For this review, take the finished solid that the model builds, in its own axes (mm). A direction names the side the tool comes from. Give positions to 0.01 mm unless a question says otherwise; leave off trailing zeros. Order: outer loops, then holes, each group sorted by start corner. A loop starts at its lowest first (then second) coordinate and runs counter-clockwise, first axis right, second up.
from build123d import *

# Parameters (mm, degrees)
SKETCH_1_W                   = 210
SKETCH_1_H                   = 60
EXTRUDE_1_DEPTH              = 12
SKETCH_2_R                   = 12.5
CUT_EXTRUDE_1_DEPTH          = 12
HOLE_WIZARD_M8_1_D           = 8.4
HOLE_WIZARD_M8_1_CBORE_D     = 15
HOLE_WIZARD_M8_1_CBORE_DEPTH = 8.6
HOLE_WIZARD_M6_2_D           = 6.4
HOLE_WIZARD_M6_2_CBORE_D     = 11
HOLE_WIZARD_M6_2_CBORE_DEPTH = 6.4
CHAMFER_1_SIZE               = 1
HOLE_WIZARD_9_0_9_1_D        = 9
SKETCH_14_W                  = 30
SKETCH_14_H                  = 20
EXTRUDE_2_DEPTH              = 12


with BuildPart() as part:
    # 草图1 → 凸台-拉伸1 (new body)
    with BuildSketch(Plane.XY):
        with Locations((105, 30)):
            Rectangle(SKETCH_1_W, SKETCH_1_H)
    extrude(amount=EXTRUDE_1_DEPTH)

    # 草图2 → 切除-拉伸1 (cut)
    with BuildSketch(Plane.XY.offset(12)):
        with Locations((105, 25)):
            Circle(SKETCH_2_R)
    extrude(amount=-CUT_EXTRUDE_1_DEPTH, mode=Mode.SUBTRACT)

    # M8 六角凹头螺钉的柱形沉头孔1 (through all)
    with Locations(Plane(origin=(0, 0, 0), x_dir=(-1, 0, 0), z_dir=(0, 0, -1))):
        with Locations((-55, 21), (-155, 21)):
            CounterBoreHole(HOLE_WIZARD_M8_1_D / 2, HOLE_WIZARD_M8_1_CBORE_D / 2, HOLE_WIZARD_M8_1_CBORE_DEPTH)

    # M6 六角凹头螺钉的柱形沉头孔2 (through all)
    with Locations(Plane.XY.offset(12)):
        with Locations((122, 42), (88, 42), (122, 8), (88, 8)):
            CounterBoreHole(HOLE_WIZARD_M6_2_D / 2, HOLE_WIZARD_M6_2_CBORE_D / 2, HOLE_WIZARD_M6_2_CBORE_DEPTH)

    # 倒角1
    chamfer_1_edges = [part.edges().sort_by_distance(p)[0] for p in [
        (210, 30, 12),
        (0, 30, 12),
        (210, 30, 0),
        (0, 30, 0),
    ]]
    chamfer(chamfer_1_edges, length=CHAMFER_1_SIZE)

    # Ø9.0 (9) 直径孔1 (through all)
    with Locations(Plane(origin=(0, 0, 0), x_dir=(-1, 0, 0), z_dir=(0, 0, -1))):
        with Locations((-192.5, 35), (-17.5, 35)):
            Hole(HOLE_WIZARD_9_0_9_1_D / 2)

    # 草图14 → 凸台-拉伸2 (add)
    with BuildSketch(Plane(origin=(0, 0, 0), x_dir=(-1, 0, 0), z_dir=(0, 0, -1))):
        with Locations((-105, -10)):
            Rectangle(SKETCH_14_W, SKETCH_14_H)
    extrude(amount=-EXTRUDE_2_DEPTH)


solid = part.part
1) We need section D-D on y = -10. Give the boundary of the cut face in (x, z).
Answer sheet:
outline: (90, 0) - (120, 0) - (120, 12) - (90, 12) - close
2) To check wall thickness, follow line 1 (Y direction, x = 122, z = 2.3); line 2 (Y direction, x = 155, z = 3.25); line 3 (Y direction, x = 127, z = 8). State the ranges of each line that lie inside material, in increasing order.
Answer sheet:
line 1: y = 0 to 4.8, 11.2 to 38.8, 45.2 to 60
line 2: y = 0 to 13.5, 28.5 to 60
line 3: y = 0 to 5.71, 10.29 to 39.71, 44.29 to 60
3) We need section B-B on y = 8. Give the boundary of the cut face in (x, z), then the cut area to 3 significant figures.
Answer sheet:
outline: (0, 1) - (1, 0) - (84.8, 0) - (84.8, 5.6) - (82.5, 5.6) - (82.5, 12) - (1, 12) - (0, 11) - close; (91.2, 0) - (118.8, 0) - (118.8, 5.6) - (116.5, 5.6) - (116.5, 12) - (93.5, 12) - (93.5, 5.6) - (91.2, 5.6) - close; (125.2, 0) - (209, 0) - (210, 1) - (210, 11) - (209, 12) - (127.5, 12) - (127.5, 5.6) - (125.2, 5.6) - close
area: 2,310 mm2
4) Clearance check with flat-ended pins moving along their axes: pin 1 (4.5 mm diameter, centred on x = 155.5, y = 17.5, fed in from -Z); pin 2 (2 mm diameter, centred on y = -8, z = 3.5, fed in from -X); pin 3 (6 mm diameter, centred on x = 166.5, z = 3.5, fed in from -Y). State where each tip first meets the part, or that it passes through.
Answer sheet:
pin 1: stops at z = 8.6
pin 2: stops at x = 90
pin 3: stops at y = 0
5) We need section A-A on x = 88. Give the boundary of the cut face in (y, z), then the cut area to 3 significant figures.
Answer sheet:
outline: (0, 0) - (4.8, 0) - (4.8, 5.6) - (2.5, 5.6) - (2.5, 12) - (0, 12) - close; (11.2, 0) - (38.8, 0) - (38.8, 5.6) - (36.5, 5.6) - (36.5, 12) - (13.5, 12) - (13.5, 5.6) - (11.2, 5.6) - close; (45.2, 0) - (60, 0) - (60, 12) - (47.5, 12) - (47.5, 5.6) - (45.2, 5.6) - close
area: 508 mm2
6) We need section C-C on x = 192.5. Give the boundary of the cut face in (y, z).
Answer sheet:
outline: (0, 0) - (30.5, 0) - (30.5, 12) - (0, 12) - close; (39.5, 0) - (60, 0) - (60, 12) - (39.5, 12) - close
7) Tool access review of faces 1 (the face through (116.505, 8.242, 8.845)), 2 (the face through (90, -10, 6)), 3 (the face through (120, -10, 6)), 4 (the face through (151.8, 17.8, 8.6)): name each direction out of +Z, -Z, +X, -X, +Y, -Y from which nothing blocks a thin tool from reaching the whole face with its end or side.
Answer sheet:
face 1: +Z
face 2: +Z, -Z, -X, -Y
face 3: +Z, -Z, +X, -Y
face 4: -Z
